```python
from build123d import *

# Parameters (mm, degrees)
SKETCH_1_W                   = 126
SKETCH_1_H                   = 110
EXTRUDE_1_DEPTH              = 5
CHAMFER_1_SIZE               = 3
HOLE_WIZARD_M5_1_D           = 5.5
HOLE_WIZARD_M5_1_CBORE_D     = 10
HOLE_WIZARD_M5_1_CBORE_DEPTH = 5.4
HOLE_WIZARD_M5_1_2_D         = 4.2
HOLE_WIZARD_M5_1_2_DEPTH     = 20
HOLE_WIZARD_M5_1_2_TIP       = 1.2618073


with BuildPart() as part:
    # 草图1 → 凸台-拉伸1 (new, symmetric)
    with BuildSketch(Plane.XY):
        Rectangle(SKETCH_1_W, SKETCH_1_H)
    extrude(amount=EXTRUDE_1_DEPTH, both=True)

    # 倒角1
    chamfer_1_edges = [part.edges().sort_by_distance(p)[0] for p in [
        (-63, 55, 0),
        (63, 55, 0),
        (63, -55, 0),
        (-63, -55, 0),
    ]]
    chamfer(chamfer_1_edges, length=CHAMFER_1_SIZE)

    # Hole Wizard M5 _1 (through all)
    with Locations(Plane.XY.offset(5)):
        with Locations((-50, 45), (-17.5, 32.5), (17.5, 32.5), (50, 45), (50, -40), (17.5, -27.5), (-50, -40)):
            CounterBoreHole(HOLE_WIZARD_M5_1_D / 2, HOLE_WIZARD_M5_1_CBORE_D / 2, HOLE_WIZARD_M5_1_CBORE_DEPTH)

    # Hole Wizard M5 _1 2
    with Locations(Plane(origin=(0, -55, 0), x_dir=(-1, 0, 0), z_dir=(0, -1, 0))):
        with Locations((20, 0), (-20, 0)):
            Hole(HOLE_WIZARD_M5_1_2_D / 2, depth=HOLE_WIZARD_M5_1_2_DEPTH)
            with Locations((0, 0, -(HOLE_WIZARD_M5_1_2_DEPTH + HOLE_WIZARD_M5_1_2_TIP / 2))):  # 118° drill point
                Cone(0, HOLE_WIZARD_M5_1_2_D / 2, HOLE_WIZARD_M5_1_2_TIP, mode=Mode.SUBTRACT)


solid = part.part
```
The model under review builds one solid part; all positions refer to its coordinate system, in mm. A direction names the side the tool comes from. Coordinates: 2 decimals unless noted, no trailing zeros. Write each loop counter-clockwise with the first axis right and the second up, starting at its lowest first coordinate (ties: lowest second). Pieces come first, ordered by that corner, then holes.
1) The part is to be moulded in two halves that separate along Y. For faces 4 (the face through (-54, 48, 2)), 5 (the face through (-19.636, -33.957, -0.016)), 6 (the face through (-1, 55, 0)), say which applies: pulls with the +Y half, pulls with the -Y half, needs draft (parallel to the pull), parting line crosses it, or undercut.
2) Machinability: for faces 1 (the face through (49.349, 49.957, 2.338)), 2 (the face through (-17.997, -44.86, -0.631)), 3 (the face through (61, -54, 0)), which of the approach directions +Z, -Z, +X, -X, +Y, -Y give a long, thin tool a straight path to every point of the face, cutting with its end or side? Answer none if there is none.
3) We need section B-B on y = -40. State the section outline as (x, z) points, then the cut area to 3 significant figures.
4) We need section A-A on y = 45. State the section outline as (x, z) points, then the cut area to 3 significant figures.
5) We need section C-C on x = -50. State the section outline as (y, z) points, then the cut area to 3 significant figures.
6) To check wall thickness, follow probe 1 along Y at (x, z) = (17.5, 1.05); probe 2 along Y at (x, z) = (-50, -2.75); probe 3 along X at (y, z) = (-38.5, 0.5). State the ranges of each line that lie inside material, in increasing order.
7) Clearance check with flat-ended pins moving along their axes: pin 1 Ø3 at (x, y) = (15, -26) entering from +Z; pin 2 Ø4.5 at (x, y) = (17.5, -27.5) entering from +Z. State where each tip first meets the part, or that it passes through.
Answer list:
1. face 4: undercut
1. face 5: pulls with the -Y half
1. face 6: pulls with the +Y half
2. face 1: +Z
2. face 2: -Y
2. face 3: +Z, -Z, +X, -Y
3. outline: (-63, -5) - (-52.75, -5) - (-52.75, -0.4) - (-55, -0.4) - (-55, 5) - (-63, 5) - close; (-47.25, -5) - (47.25, -5) - (47.25, -0.4) - (45, -0.4) - (45, 5) - (-45, 5) - (-45, -0.4) - (-47.25, -0.4) - close; (52.75, -5) - (63, -5) - (63, 5) - (55, 5) - (55, -0.4) - (52.75, -0.4) - close; hole circle Ø4.2 at (-20, 0); hole circle Ø4.2 at (20, 0)
3. area: 1,070 mm2
4. outline: (-63, -5) - (-52.75, -5) - (-52.75, -0.4) - (-55, -0.4) - (-55, 5) - (-63, 5) - close; (-47.25, -5) - (47.25, -5) - (47.25, -0.4) - (45, -0.4) - (45, 5) - (-45, 5) - (-45, -0.4) - (-47.25, -0.4) - close; (52.75, -5) - (63, -5) - (63, 5) - (55, 5) - (55, -0.4) - (52.75, -0.4) - close
4. area: 1,100 mm2
5. outline: (-55, -5) - (-42.75, -5) - (-42.75, -0.4) - (-45, -0.4) - (-45, 5) - (-55, 5) - close; (-37.25, -5) - (42.25, -5) - (42.25, -0.4) - (40, -0.4) - (40, 5) - (-35, 5) - (-35, -0.4) - (-37.25, -0.4) - close; (47.75, -5) - (55, -5) - (55, 5) - (50, 5) - (50, -0.4) - (47.75, -0.4) - close
5. area: 941 mm2
6. probe 1: y = -55 to -32.5, -22.5 to 27.5, 37.5 to 55
6. probe 2: y = -55 to -42.75, -37.25 to 42.25, 47.75 to 55
6. probe 3: x = -63 to -54.77, -45.23 to -22.04, -17.96 to 17.96, 22.04 to 45.23, 54.77 to 63
7. pin 1: stops at z = -0.4
7. pin 2: passes through
